```python
from build123d import *

# Parameters (mm, degrees)
SKETCH1_W           = 5
SKETCH1_H           = 18
BOSS_EXTRUDE1_DEPTH = 6
SKETCH2_R           = 1.3
CUT_EXTRUDE1_DEPTH  = 10
SKETCH3_R           = 2.3
CUT_EXTRUDE2_DEPTH  = 3


with BuildPart() as part:
    # Sketch1 → Boss-Extrude1 (new body)
    with BuildSketch(Plane(origin=(0, 0, 0), x_dir=(1, 0, 0), z_dir=(0, 1, 0))):
        Rectangle(SKETCH1_W, SKETCH1_H)
    extrude(amount=BOSS_EXTRUDE1_DEPTH)

    # Sketch2 → Cut-Extrude1 (cut)
    with BuildSketch(Plane.ZY.offset(2.5)):
        with Locations((6, 3)):
            Circle(SKETCH2_R)
        with Locations((-6, 3)):
            Circle(SKETCH2_R)
    extrude(amount=-CUT_EXTRUDE1_DEPTH, mode=Mode.SUBTRACT)

    # Sketch3 → Cut-Extrude2 (cut)
    with BuildSketch(Plane.ZY.offset(2.5)):
        with Locations((-6, 3)):
            Circle(SKETCH3_R)
        with Locations((6, 3)):
            Circle(SKETCH3_R)
    extrude(amount=-CUT_EXTRUDE2_DEPTH, mode=Mode.SUBTRACT)


solid = part.part
```
Part model, mm, in its own coordinate system. A direction names the side the tool comes from. Give positions to 0.01 mm unless a question says otherwise; leave off trailing zeros. Write each loop counter-clockwise with the first axis right and the second up, starting at its lowest first coordinate (ties: lowest second). Pieces come first, ordered by that corner, then holes. Notation, with made-up numbers: (47.25, 16) -> (98.25, 16) arc R21 cw to (98.25, 31) -> close; hole circle Ø10 at (-26, 61.25). An arc over 180 degrees is marked (long way). Put each result on its own line as item: value. Start each with the question number.
Item 1: Cut at B-B (y = 3). List the corners of the cut face in (x, z), then the cut area to 3 significant figures.
Item 2: Which spindle directions (+Z, -Z, +X, -X, +Y, -Y) get a long thin tool onto all of the face, cutting with end or side? Do faces 4 (the face through (0.5, 3, 8)), 5 (the face through (-2.5, 3, 0)). Say none if no direction does.
Item 3: Cut at C-C (x = -2). List the corners of the cut face in (y, z).
Item 4: Pull direction Z, two halves, no side cores. Call faces 1 (the face through (0, 6, 0)), 2 (the face through (1.49, 3.39, 7.24)), 3 (the face through (0, 3, -9)): pulls with the +Z half, pulls with the -Z half, needs draft (parallel to the pull), parting line crosses it, or undercut.
Item 5: Pin check, flat tip, straight feed: pin 1 Ø3.5 at (y, z) = (3, 6) entering from -X. Stop position of the tip, or through.
Item 6: Wall check: L1, parallel to Y at x = 1.35, z = 6; L2, parallel to Y at x = -0.2, z = 6; L3, parallel to Z at x = -1.5, y = 4.4. Give the ranges that are in metal, low to high. Write a range as [from, to].
Item 7: Cut at A-A (z = -6). List the corners of the cut face in (x, y).
Item 8: Cut at D-D (z = 5.75). List the corners of the cut face in (x, y).
Answer list:
1. outline: (-2.5, -9) -> (2.5, -9) -> (2.5, -7.3) -> (0.5, -7.3) -> (0.5, -8.3) -> (-2.5, -8.3) -> close; (-2.5, -3.7) -> (0.5, -3.7) -> (0.5, -4.7) -> (2.5, -4.7) -> (2.5, 4.7) -> (0.5, 4.7) -> (0.5, 3.7) -> (-2.5, 3.7) -> close; (-2.5, 8.3) -> (0.5, 8.3) -> (0.5, 7.3) -> (2.5, 7.3) -> (2.5, 9) -> (-2.5, 9) -> close
1. area: 52.0 mm2
2. face 4: -X
2. face 5: +Z, -Z, -X, +Y, -Y
3. outline: (0, -9) -> (6, -9) -> (6, 9) -> (0, 9) -> close; hole circle Ø4.6 at (3, -6); hole circle Ø4.6 at (3, 6)
4. face 1: needs draft
4. face 2: undercut
4. face 3: pulls with the -Z half
5. pin 1: stops at x = 0.5
6. L1: y = [0, 1.7], [4.3, 6]
6. L2: y = [0, 0.7], [5.3, 6]
6. L3: z = [-9, -7.82], [-4.18, 4.18], [7.82, 9]
7. outline: (-2.5, 0) -> (2.5, 0) -> (2.5, 1.7) -> (0.5, 1.7) -> (0.5, 0.7) -> (-2.5, 0.7) -> close; (-2.5, 5.3) -> (0.5, 5.3) -> (0.5, 4.3) -> (2.5, 4.3) -> (2.5, 6) -> (-2.5, 6) -> close
8. outline: (-2.5, 0) -> (2.5, 0) -> (2.5, 1.72) -> (0.5, 1.72) -> (0.5, 0.71) -> (-2.5, 0.71) -> close; (-2.5, 5.29) -> (0.5, 5.29) -> (0.5, 4.28) -> (2.5, 4.28) -> (2.5, 6) -> (-2.5, 6) -> close
